Design review of the part built by this model. Coordinates are the model's own, in mm. A direction names the side the tool comes from. Give positions to 0.01 mm unless a question says otherwise; leave off trailing zeros. Loops run counter-clockwise (first coordinate to the right, second up) from the corner with the lowest first, then second, coordinate; pieces in that order, holes last. Notation, with made-up numbers: (45.25, -25) -> (86.25, -25) arc R21 ccw to (86.25, 6) -> close; hole circle Ø4 at (53.5, 50.5). An arc over 180 degrees is marked (long way). Use CSV: the item, a comma, the result in double quotes. Start each with the question number.
Item 1: Clearance check with flat-ended pins moving along their axes: pin 1 (9.5 mm diameter, centred on x = -15, y = -38.5, fed in from -Z); pin 2 (4 mm diameter, centred on x = 37, y = 37, fed in from +Z); pin 3 (0.5 mm diameter, centred on x = 3, z = 8.5, fed in from +Y). State where each tip first meets the part, or that it passes through.
Item 2: We need section C-C (x = 4.5). State the section outline as (y, z) points, plus the area to 3 significant figures.
Item 3: We need section A-A (x = -14). State the section outline as (y, z) points.
Item 4: The part is to be moulded in two halves that separate along Y. For faces 1 (the face through (-11.231, 44.323, 2.958)), 2 (the face through (-1, 0, 9)), 3 (the face through (-13.54, -35.53, 6.99)), 4 (the face through (1, 55, 4)), say which applies: +Y half, -Y half, draft (parallel to the pull), parting line (faces both ways), or undercut.
Item 5: For faces 5 (the face through (16.769, 44.323, 2.958)), 6 (the face through (49, 53, 4)), list the 3-axis set-ups (+Z, -Z, +X, -X, +Y, -Y) from which the entire face can be reached by the end or side of a thin tool; tool diameter is ignored.
Item 6: We need section B-B (y = -39). State the section outline as (x, z) points, plus the area to 3 significant figures.
Item 7: Wall thickness on line 1 along Y through (x, z) = (-14, 1.4); line 2 along Y through (x, z) = (14, 6.5); line 3 along X through (y, z) = (39, 4.65): over which ranges is each line inside the solid? List them lowest first. Write a range as from..to.
from build123d import *

# Parameters (mm, degrees)
BOSS_EXTRUDE1_DEPTH = 8
SKETCH2_W           = 88
SKETCH2_H           = 58
BOSS_EXTRUDE2_DEPTH = 1
SKETCH4_R           = 6
CUT_EXTRUDE1_DEPTH  = 6
SKETCH5_R           = 3.5
CUT_EXTRUDE2_DEPTH  = 6


with BuildPart() as part:
    # Sketch1 → Boss-Extrude1 (new body)
    with BuildSketch(Plane.XY):
        with BuildLine():
            Line((-45, -55), (45, -55))
            ThreePointArc((45, -55), (48.535533906, -53.535533906), (50, -50))
            Line((50, -50), (50, 50))
            ThreePointArc((50, 50), (48.535533906, 53.535533906), (45, 55))
            Line((45, 55), (-45, 55))
            ThreePointArc((-45, 55), (-48.535533906, 53.535533906), (-50, 50))
            Line((-50, 50), (-50, -50))
            ThreePointArc((-50, -50), (-48.535533906, -53.535533906), (-45, -55))
        make_face()
    extrude(amount=BOSS_EXTRUDE1_DEPTH)

    # Sketch2 → Boss-Extrude2 (add)
    with BuildSketch(Plane.XY.offset(8)):
        Rectangle(SKETCH2_W, SKETCH2_H)
    extrude(amount=BOSS_EXTRUDE2_DEPTH)

    # Sketch4 → Cut-Extrude1 (cut)
    with BuildSketch(Plane(origin=(0, 0, 0), x_dir=(-1, 0, 0), z_dir=(0, 0, -1))):
        with Locations((-14, -39)):
            Circle(SKETCH4_R)
        with Locations((14, -39)):
            Circle(SKETCH4_R)
        with Locations(Location((14, 39, 0), (0, 0, 180))):
            Circle(SKETCH4_R)
        with Locations(Location((-14, 39, 0), (0, 0, 180))):
            Circle(SKETCH4_R)
    extrude(amount=-CUT_EXTRUDE1_DEPTH, mode=Mode.SUBTRACT)

    # Sketch5 → Cut-Extrude2 (cut)
    with BuildSketch(Plane(origin=(0, 0, 6), x_dir=(-1, 0, 0), z_dir=(0, 0, -1))):
        with Locations((-14, 39)):
            Circle(SKETCH5_R)
        with Locations((14, 39)):
            Circle(SKETCH5_R)
        with Locations((14, -39)):
            Circle(SKETCH5_R)
        with Locations((-14, -39)):
            Circle(SKETCH5_R)
    extrude(amount=-CUT_EXTRUDE2_DEPTH, mode=Mode.SUBTRACT)


solid = part.part
Results found:
1,pin 1,"z = 6"
1,pin 2,"z = 8"
1,pin 3,"y = 29"
2,outline,"(-55, 0) -> (55, 0) -> (55, 8) -> (29, 8) -> (29, 9) -> (-29, 9) -> (-29, 8) -> (-55, 8) -> close"
2,area,"938 mm²"
3,outline,"(-55, 0) -> (-45, 0) -> (-45, 6) -> (-42.5, 6) -> (-42.5, 8) -> (-55, 8) -> close; (-35.5, 6) -> (-33, 6) -> (-33, 0) -> (33, 0) -> (33, 6) -> (35.5, 6) -> (35.5, 8) -> (29, 8) -> (29, 9) -> (-29, 9) -> (-29, 8) -> (-35.5, 8) -> close; (42.5, 6) -> (45, 6) -> (45, 0) -> (55, 0) -> (55, 8) -> (42.5, 8) -> close"
4,face 1,"undercut"
4,face 2,"draft"
4,face 3,"undercut"
4,face 4,"+Y half"
5,face 5,"-Z"
5,face 6,"+Z, -Z, +X, +Y"
6,outline,"(-50, 0) -> (-20, 0) -> (-20, 6) -> (-17.5, 6) -> (-17.5, 8) -> (-50, 8) -> close; (-10.5, 6) -> (-8, 6) -> (-8, 0) -> (8, 0) -> (8, 6) -> (10.5, 6) -> (10.5, 8) -> (-10.5, 8) -> close; (17.5, 6) -> (20, 6) -> (20, 0) -> (50, 0) -> (50, 8) -> (17.5, 8) -> close"
6,area,"628 mm²"
7,line 1,"-55..-45, -33..33, 45..55"
7,line 2,"-55..-42.5, -35.5..35.5, 42.5..55"
7,line 3,"-50..-20, -8..8, 20..50"
